Check sheet for the modelled part. Datum: model origin and axes. Units: mm. Face numbers are marked on the shaded views. A direction names the side the tool comes from. Give positions to 0.01 mm unless a question says otherwise; leave off trailing zeros. Order: outer loops, then holes, each group sorted by start corner. A loop starts at its lowest first (then second) coordinate and runs counter-clockwise, first axis right, second up.
```python
from build123d import *

# Parameters (mm, degrees)
SKETCH1_W           = 50
SKETCH1_H           = 6
BOSS_EXTRUDE1_DEPTH = 6
SKETCH2_R           = 3
BOSS_EXTRUDE2_DEPTH = 6
SKETCH3_W           = 10
SKETCH3_H           = 6
BOSS_EXTRUDE3_DEPTH = 3
SKETCH4_W           = 6
SKETCH4_H           = 6
CUT_EXTRUDE1_DEPTH  = 20
SKETCH5_W           = 8
SKETCH5_H           = 6
BOSS_EXTRUDE4_DEPTH = 2
SKETCH6_W           = 3
SKETCH6_H           = 10
BOSS_EXTRUDE5_DEPTH = 8


with BuildPart() as part:
    # Sketch1 → Boss-Extrude1 (new body)
    with BuildSketch(Plane.XY):
        Rectangle(SKETCH1_W, SKETCH1_H)
    extrude(amount=BOSS_EXTRUDE1_DEPTH)

    # Sketch2 → Boss-Extrude2 (add)
    with BuildSketch(Plane.XZ.offset(3)):
        with Locations(Location((-10, 3, 0), (0, 0, 270))):
            Circle(SKETCH2_R)
    extrude(amount=BOSS_EXTRUDE2_DEPTH)

    # Sketch3 → Boss-Extrude3 (add)
    with BuildSketch(Plane.ZY.offset(25)):
        with Locations((3, 0)):
            Rectangle(SKETCH3_W, SKETCH3_H)
    extrude(amount=-BOSS_EXTRUDE3_DEPTH)

    # Sketch4 → Cut-Extrude1 (cut)
    with BuildSketch(Plane(origin=(25, 0, 0), x_dir=(0, 0, -1), z_dir=(1, 0, 0))):
        with Locations((-3, 0)):
            Rectangle(SKETCH4_W, SKETCH4_H)
    extrude(amount=-CUT_EXTRUDE1_DEPTH, mode=Mode.SUBTRACT)

    # Sketch5 → Boss-Extrude4 (add)
    with BuildSketch(Plane(origin=(5, 0, 0), x_dir=(0, 0, -1), z_dir=(1, 0, 0))):
        with Locations((-3, 0)):
            Rectangle(SKETCH5_W, SKETCH5_H)
    extrude(amount=BOSS_EXTRUDE4_DEPTH)

    # Sketch6 → Boss-Extrude5 (add)
    with BuildSketch(Plane(origin=(0, 3, 0), x_dir=(1, 0, 0), z_dir=(0, 1, 0))):
        with Locations((-23.5, -3)):
            Rectangle(SKETCH6_W, SKETCH6_H)
    extrude(amount=BOSS_EXTRUDE5_DEPTH)


solid = part.part
```
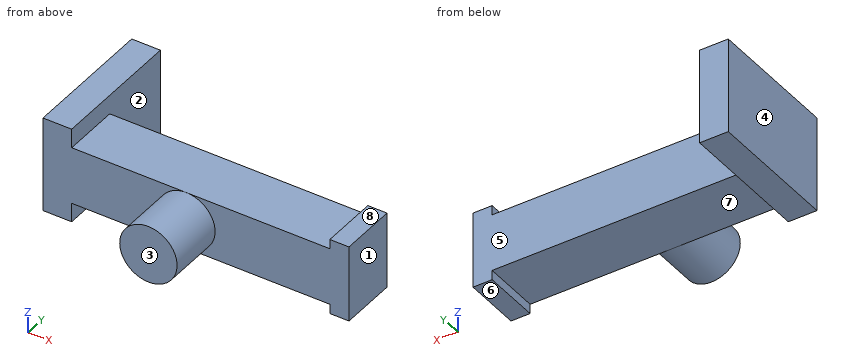
(1) Sectioned sample at B-B (z = 3). Enter the section's corners in (x, y), plus the area to 3 significant figures.
(2) Sectioned sample at C-C (x = -11.5). Enter the section's corners in (y, z), plus the area to 3 significant figures.
(3) Thickness scan on L1, parallel to X at y = 3.5, z = 5.5; L2, parallel to Y at x = 5.5, z = 1; L3, parallel to Y at x = -11.5, z = 1. Record the ranges inside material, lowest first.
(4) Go/stop test with flat-tipped pins: P1, Ø8, axis at x = 3, y = -5.5, coming from the -Z side; P2, Ø3, axis at x = -16, z = 2, coming from the -Y side; P3, Ø3, axis at x = -4, y = -1.5, coming from the -Z side; P4, Ø5, axis at y = -4, z = 2, coming from the +X side. Record where each tip stops, or that it passes through.
(5) Sectioned sample at A-A (y = -0.5). Enter the section's corners in (x, z), plus the area to 3 significant figures.
(6) Release check for a two-part mould opening along X. For the marked faces 1, 2, 3 and 4 record: released by +X, released by -X, zero draft, split by the parting line, or undercut.
(7) Tool access check on the marked faces 5, 6, 7 and 8. Record the directions out of +Z, -Z, +X, -X, +Y, -Y that give a thin tool (end or side, any length) a straight path to the whole face; none if there is none.
(8) Sectioned sample at D-D (z = 0.75). Enter the section's corners in (x, y), plus the area to 3 significant figures.
Values follow:
1. outline: (-25, -3) - (-13, -3) - (-13, -9) - (-7, -9) - (-7, -3) - (7, -3) - (7, 3) - (-22, 3) - (-22, 11) - (-25, 11) - close
1. area: 252 mm2
2. outline: (-9, 0.4) - (-3, 0.4) - (-3, 0) - (3, 0) - (3, 6) - (-3, 6) - (-3, 5.6) - (-9, 5.6) - close
2. area: 67.2 mm2
3. L1: x = -25 to -22
3. L2: y = -3 to 3
3. L3: y = -9 to 3
4. P1: stops at z = -1
4. P2: stops at y = -3
4. P3: stops at z = 0
4. P4: stops at x = 7
5. outline: (-25, -2) - (-22, -2) - (-22, 0) - (5, 0) - (5, -1) - (7, -1) - (7, 7) - (5, 7) - (5, 6) - (-22, 6) - (-22, 8) - (-25, 8) - close
5. area: 208 mm2
6. face 1: released by +X
6. face 2: undercut
6. face 3: zero draft
6. face 4: released by -X
7. face 5: +Z, -Z, +X, +Y
7. face 6: -Z, +X, +Y, -Y
7. face 7: -Z, +Y, -Y
7. face 8: +Z, +X, +Y, -Y
8. outline: (-25, -3) - (-11.98, -3) - (-11.98, -9) - (-8.02, -9) - (-8.02, -3) - (7, -3) - (7, 3) - (-22, 3) - (-22, 11) - (-25, 11) - close
8. area: 240 mm2
